```python
from build123d import *

# Parameters (mm, degrees)
SKETCH1_W                                    = 50
SKETCH1_H                                    = 12
BOSS_EXTRUDE1_DEPTH                          = 22.5
M8X1_0_TAPPED_HOLE1_D                        = 7
HEX_SOCKET_CAP_SCREW_HOLE_TYPE_1_D           = 5.5
HEX_SOCKET_CAP_SCREW_HOLE_TYPE_1_CBORE_D     = 10
HEX_SOCKET_CAP_SCREW_HOLE_TYPE_1_CBORE_DEPTH = 35
CHAMFER1_SIZE                                = 2


with BuildPart() as part:
    # Sketch1 → Boss-Extrude1 (new, symmetric)
    with BuildSketch(Plane.XY):
        Rectangle(SKETCH1_W, SKETCH1_H)
    extrude(amount=BOSS_EXTRUDE1_DEPTH, both=True)

    # M8x1.0 Tapped Hole1 (through all)
    with Locations(Plane(origin=(0, 6, 0), x_dir=(1, 0, 0), z_dir=(0, 1, 0))):
        with Locations((0, -10)):
            Hole(M8X1_0_TAPPED_HOLE1_D / 2)

    # Hex socket cap screw hole type 1 (through all)
    with Locations(Plane.XY.offset(22.5)):
        with Locations((-17.5, 0), (17.5, 0)):
            CounterBoreHole(HEX_SOCKET_CAP_SCREW_HOLE_TYPE_1_D / 2, HEX_SOCKET_CAP_SCREW_HOLE_TYPE_1_CBORE_D / 2, HEX_SOCKET_CAP_SCREW_HOLE_TYPE_1_CBORE_DEPTH)

    # Chamfer1
    chamfer1_edges = [part.edges().sort_by_distance(p)[0] for p in [
        (25, 0, 22.5),
        (-25, 0, 22.5),
    ]]
    chamfer(chamfer1_edges, length=CHAMFER1_SIZE)


solid = part.part
```
The model under review builds one solid part; all positions refer to its coordinate system, in mm. A direction names the side the tool comes from. Round coordinates to 2 decimals unless told otherwise and drop trailing zeros. Loops run counter-clockwise (first coordinate to the right, second up) from the corner with the lowest first, then second, coordinate; pieces in that order, holes last. Notation, with made-up numbers: (22, -25.5) - (67, -25.5) arc R13 ccw to (67, -7.5) - close; hole circle Ø2 at (-38.75, 22). An arc over 180 degrees is marked (long way). Write each question's results on one line, items separated by ' | '. Start each with the question number.
Q1. Insertion check: P1, Ø6, axis at x = -17.5, y = 0, coming from the +Z side. The pin has a flat end and moves straight along its axis. Give the tip position at first contact, or say it passes through.
Q2. Take a section at A-A on z = 10. Give the boundary of the cut face in (x, y).
Q3. Take a section at D-D on z = -16.5. Give the boundary of the cut face in (x, y).
Q4. Wall thickness on line 1 along X through (y, z) = (-0.5, 5.5); line 2 along X through (y, z) = (-1, -0.5); line 3 along Z through (x, y) = (-22, 0.5): over which ranges is each line inside the solid? List them lowest first. Write a range as [from, to].
Q5. Take a section at B-B on x = 0. Give the boundary of the cut face in (y, z).
Q6. Take a section at C-C on y = 0. Give the boundary of the cut face in (x, z).
Q7. Draft analysis for pull direction X (two halves, no side actions). For faces 1 (the flat face through (-24, -0.1, 21.5)), 2 (the flat face through (25, 0, -1)), 3 (the cylindrical face through (-22.495, 0.22, 5.245)), 4 (the cylindrical face through (0.759, -0.084, 13.417)), state which applies: pulls with the +X half, pulls with the -X half, needs draft (parallel to the pull), parting line crosses it, or undercut.
Q8. Tool access review of faces 5 (the flat face through (24, -0.1, 21.5)), 6 (the cylindrical face through (12.505, 0.22, 5.245)): name each direction out of +Z, -Z, +X, -X, +Y, -Y from which nothing blocks a thin tool from reaching the whole face with its end or side.
Data:
1) P1: stops at z = -12.5
2) outline: (-25, -6) - (-3.5, -6) - (-3.5, 6) - (-25, 6) - close; (3.5, -6) - (25, -6) - (25, 6) - (3.5, 6) - close; hole circle Ø10 at (-17.5, 0); hole circle Ø10 at (17.5, 0)
3) outline: (-25, -6) - (25, -6) - (25, 6) - (-25, 6) - close; hole circle Ø5.5 at (-17.5, 0); hole circle Ø5.5 at (17.5, 0)
4) line 1: x = [-25, -22.47], [-12.53, 12.53], [22.47, 25] | line 2: x = [-25, -22.4], [-12.6, 12.6], [22.4, 25] | line 3: z = [-22.5, -12.5]
5) outline: (-6, -22.5) - (6, -22.5) - (6, 6.5) - (-6, 6.5) - close; (-6, 13.5) - (6, 13.5) - (6, 22.5) - (-6, 22.5) - close
6) outline: (-25, -22.5) - (-20.25, -22.5) - (-20.25, -12.5) - (-22.5, -12.5) - (-22.5, 22.5) - (-23, 22.5) - (-25, 20.5) - close; (-14.75, -22.5) - (14.75, -22.5) - (14.75, -12.5) - (12.5, -12.5) - (12.5, 22.5) - (-12.5, 22.5) - (-12.5, -12.5) - (-14.75, -12.5) - close; (20.25, -22.5) - (25, -22.5) - (25, 20.5) - (23, 22.5) - (22.5, 22.5) - (22.5, -12.5) - (20.25, -12.5) - close; hole circle Ø7 at (0, 10)
7) face 1: pulls with the -X half | face 2: pulls with the +X half | face 3: undercut | face 4: undercut
8) face 5: +Z, +X, +Y, -Y | face 6: +Z
